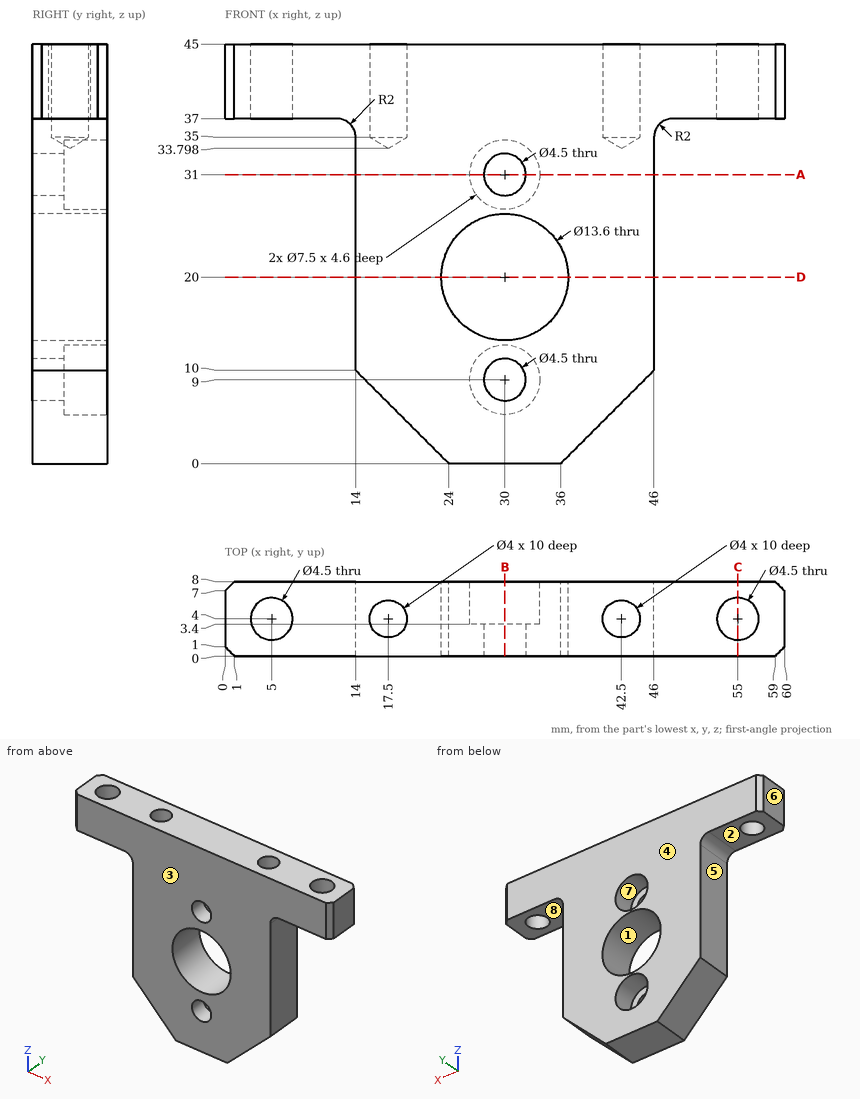
The figure shows three views and two pictorial views of one solid part (mm, origin at its lowest corner). Answer the questions. A direction names the side the tool comes from. Coordinates: 2 decimals unless noted, no trailing zeros. Write each loop counter-clockwise with the first axis right and the second up, starting at its lowest first coordinate (ties: lowest second). Pieces come first, ordered by that corner, then holes. Notation, with made-up numbers: (71, 12.25) -> (124, 12.25) arc R15 ccw to (124, 19.25) -> close; hole circle Ø7 at (40, 62.25). An arc over 180 degrees is marked (long way). Answer as a JSON object with one key per item and string values.
Q1. The part is cut by section D-D on z = 20. Give the vertices of the cut face in (x, y), then the cut area to 3 significant figures.
The answers:
{"outline": "(14, 0) -> (23.2, 0) -> (23.2, 8) -> (14, 8) -> close; (36.8, 0) -> (46, 0) -> (46, 8) -> (36.8, 8) -> close", "area": "147 mm2"}
Q2. The part is cut by section A-A on z = 31. Give the vertices of the cut face in (x, y), then the cut area to 3 significant figures.
The answers:
{"outline": "(14, 0) -> (27.75, 0) -> (27.75, 3.4) -> (26.25, 3.4) -> (26.25, 8) -> (14, 8) -> close; (32.25, 0) -> (46, 0) -> (46, 8) -> (33.75, 8) -> (33.75, 3.4) -> (32.25, 3.4) -> close", "area": "206 mm2"}
Q3. The part is cut by section B-B on x = 30. Give the vertices of the cut face in (y, z), then the cut area to 3 significant figures.
The answers:
{"outline": "(0, 0) -> (8, 0) -> (8, 5.25) -> (3.4, 5.25) -> (3.4, 6.75) -> (0, 6.75) -> close; (0, 11.25) -> (3.4, 11.25) -> (3.4, 12.75) -> (8, 12.75) -> (8, 13.2) -> (0, 13.2) -> close; (0, 26.8) -> (8, 26.8) -> (8, 27.25) -> (3.4, 27.25) -> (3.4, 28.75) -> (0, 28.75) -> close; (0, 33.25) -> (3.4, 33.25) -> (3.4, 34.75) -> (8, 34.75) -> (8, 45) -> (0, 45) -> close", "area": "152 mm2"}
Q4. Consider line 1 (X direction, y = 4, z = 35); line 2 (X direction, y = 1, z = 31); line 3 (Y direction, x = 42.5, z = 41.5). Determine where each line is inside the solid, lowest interval first. Write a range as [from, to].
The answers:
{"line 1": "x = [14, 15.5], [19.5, 40.5], [44.5, 46]", "line 2": "x = [14, 27.75], [32.25, 46]", "line 3": "y = [0, 2], [6, 8]"}
Q5. Flat-ended cylindrical pins translate along their axes: pin 1 Ø3 at (x, y) = (46, 6.5) entering from -Z; pin 2 Ø2 at (y, z) = (3, 16.5) entering from +X; pin 3 Ø2 at (x, z) = (31.5, 7) entering from +Y. Find the tip coordinate at first contact, or state that the pin passes through.
The answers:
{"pin 1": "stops at z = 8.5", "pin 2": "stops at x = 46", "pin 3": "stops at y = 3.4"}
Q6. A tool of negligible diameter and unlimited length cuts with its end or side. For the marked faces 4, 5, 6, 7 and 8, from which of +Z, -Z, +X, -X, +Y, -Y can it reach the whole face along a straight path? Write none if from no direction.
The answers:
{"face 4": "+Z, -Z, +X, -X, +Y", "face 5": "-Z, -X, +Y, -Y", "face 6": "+Z, -Z, -X, +Y, -Y", "face 7": "+Y", "face 8": "-Z, +X, +Y, -Y"}
Q7. The part is cut by section C-C on x = 55. Give the vertices of the cut face in (y, z), then the cut area to 3 significant figures.
The answers:
{"outline": "(0, 37) -> (1.75, 37) -> (1.75, 45) -> (0, 45) -> close; (6.25, 37) -> (8, 37) -> (8, 45) -> (6.25, 45) -> close", "area": "28.0 mm2"}
Q8. Determine the mould class of the marked faces 1, 2 and 3 for opening direction Z: pulls with the +Z half, pulls with the -Z half, needs draft (parallel to the pull), parting line crosses it, or undercut.
The answers:
{"face 1": "undercut", "face 2": "pulls with the -Z half", "face 3": "needs draft"}
